from build123d import *

# Parameters (mm, degrees)
BOSS_EXTRUDE1_DEPTH = 1716
SKETCH2_R           = 6.5
CUT_EXTRUDE1_DEPTH  = 1719.853105998
LPATTERN1_COUNT     = 2
LPATTERN1_PITCH     = 928


with BuildPart() as part:
    # Sketch1 → Boss-Extrude1 (new body)
    with BuildSketch(Plane.XY):
        with BuildLine():
            Line((12, 0), (58, 0))
            ThreePointArc((58, 0), (66.485281374, 3.514718626), (70, 12))
            Line((70, 12), (70, 58))
            ThreePointArc((70, 58), (66.485281374, 66.485281374), (58, 70))
            Line((58, 70), (12, 70))
            ThreePointArc((12, 70), (3.514718626, 66.485281374), (0, 58))
            Line((0, 58), (0, 12))
            ThreePointArc((0, 12), (3.514718626, 3.514718626), (12, 0))
        make_face()
        with BuildLine():
            Line((12, 6), (58, 6))
            ThreePointArc((58, 6), (62.242640687, 7.757359313), (64, 12))
            Line((64, 12), (64, 58))
            ThreePointArc((64, 58), (62.242640687, 62.242640687), (58, 64))
            Line((58, 64), (12, 64))
            ThreePointArc((12, 64), (7.757359313, 62.242640687), (6, 58))
            Line((6, 58), (6, 12))
            ThreePointArc((6, 12), (7.757359313, 7.757359313), (12, 6))
        make_face(mode=Mode.SUBTRACT)
    extrude(amount=BOSS_EXTRUDE1_DEPTH)

    # Sketch2 → Cut-Extrude1 (cut, through all)
    with BuildSketch(Plane.ZY):
        with Locations((248, 26)):
            Circle(SKETCH2_R)
        with Locations((540, 26)):
            Circle(SKETCH2_R)
    cut_extrude1 = extrude(amount=-CUT_EXTRUDE1_DEPTH, mode=Mode.SUBTRACT)

    # LPattern1: Cut-Extrude1 ×2
    with Locations(*[(0, 0, i * LPATTERN1_PITCH) for i in range(1, LPATTERN1_COUNT)]):
        add(cut_extrude1, mode=Mode.SUBTRACT)


solid = part.part
The model under review builds one solid part; all positions refer to its coordinate system, in mm. A direction names the side the tool comes from. Give positions to 0.01 mm unless a question says otherwise; leave off trailing zeros. Order: outer loops, then holes, each group sorted by start corner. A loop starts at its lowest first (then second) coordinate and runs counter-clockwise, first axis right, second up. Notation, with made-up numbers: M -4,29 L 14,29 A21 ccw 14,61 Z; hole C -2,-17.5 d2. An arc over 180 degrees is marked long. Answer in a Markdown table with one row per item. Add a question column.
1. Add section A-A on y = 46. State the section outline as (x, z) points.
2. Add section C-C on z = 455.5. State the section outline as (x, y) points.
3. Machinability: for faces 5 (the flat face through (35, 4, 1716)), 6 (the flat face through (35, 6, 846)), which of the approach directions +Z, -Z, +X, -X, +Y, -Y give a long, thin tool a straight path to every point of the face, cutting with its end or side? Answer none if there is none.
4. To check wall thickness, follow line 1 along X through (y, z) = (14, 739); line 2 along Y through (x, z) = (1.45, 1176). State the ranges of each line that lie inside material, in increasing order.
5. Mouldability with a two-part tool opening along X and no side actions: class faces 1 (the flat face through (70, 35, 846)), 2 (the flat face through (0, 35, 846)), 3 (the flat face through (6, 35, 846)), 4 (the flat face through (35, 0, 846)) as released by +X, released by -X, zero draft, split by the parting line, or undercut.
6. For pin 1 Ø11.5 at (y, z) = (26, 248) entering from +X; pin 2 Ø3 at (x, z) = (9, 1398) entering from -Y, all flat-tipped, find the tip position at first contact; note any pin that passes through.
The answers:
| question | item | result |
|---|---|---|
| 1 | outline | M 0,0 L 6,0 L 6,1716 L 0,1716 Z; M 64,0 L 70,0 L 70,1716 L 64,1716 Z |
| 2 | outline | M 0,12 A12 ccw 12,0 L 58,0 A12 ccw 70,12 L 70,58 A12 ccw 58,70 L 12,70 A12 ccw 0,58 Z; hole M 6,12 A6 ccw 12,6 L 58,6 A6 ccw 64,12 L 64,58 A6 ccw 58,64 L 12,64 A6 ccw 6,58 Z |
| 3 | face 5 | +Z, +X, -X, +Y, -Y |
| 3 | face 6 | +Z, -Z |
| 4 | line 1 | 0 to 6, 64 to 70 |
| 4 | line 2 | 6.28 to 19.5, 32.5 to 63.72 |
| 5 | face 1 | released by +X |
| 5 | face 2 | released by -X |
| 5 | face 3 | undercut |
| 5 | face 4 | zero draft |
| 6 | pin 1 | through |
| 6 | pin 2 | y = 0.09 |
